Part print with two shaded views. Sizes in mm from the minimum x, y, z corner. A direction names the side the tool comes from. Give positions to 0.01 mm unless a question says otherwise; leave off trailing zeros. Write each loop counter-clockwise with the first axis right and the second up, starting at its lowest first coordinate (ties: lowest second). Pieces come first, ordered by that corner, then holes.
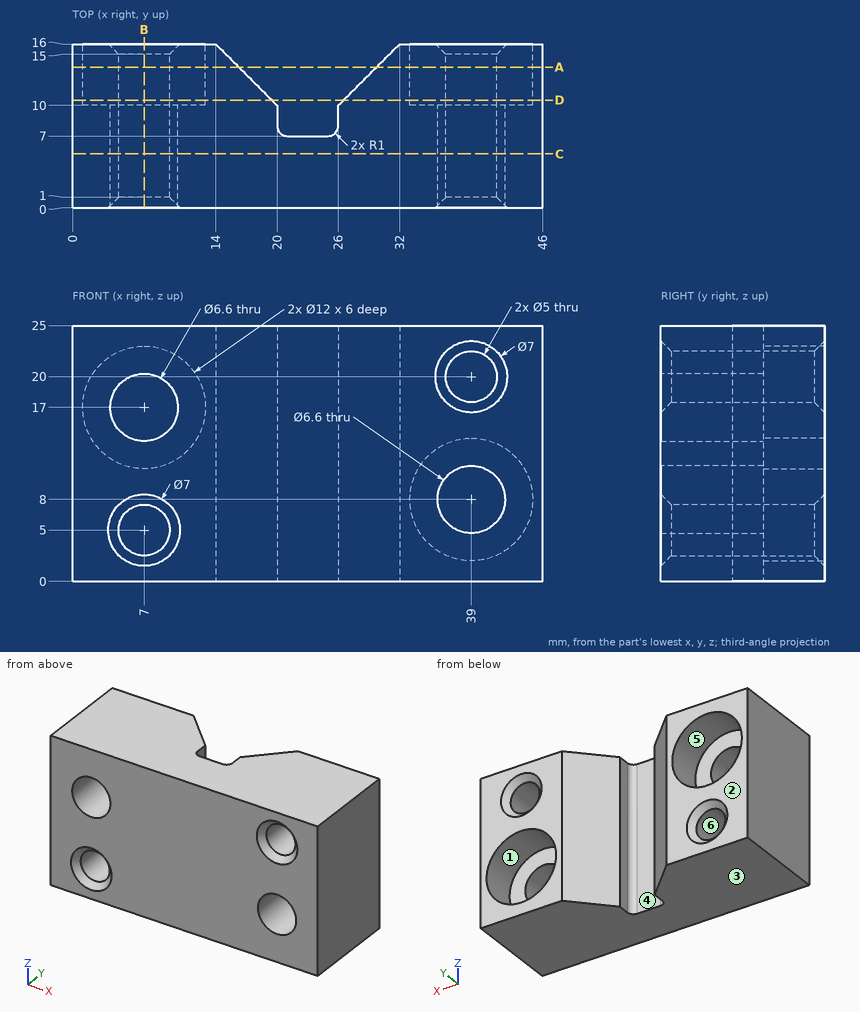
1) Two-plate mould, pull along Z, no slides. Class the marked faces 1, 2 and 3: +Z half, -Z half, draft (parallel to the pull), parting line (faces both ways), or undercut.
Answers follow:
face 1: undercut
face 2: draft
face 3: -Z half
2) Pin check, flat tips, straight feed: pin 1 Ø2 at (x, z) = (23, 14.5) entering from +Y; pin 2 Ø3 at (x, z) = (25.5, 22) entering from +Y; pin 3 Ø6 at (x, z) = (18.5, 4) entering from +Y. Stop position of each tip, or through.
Answers follow:
pin 1: stops at y = 7
pin 2: stops at y = 11
pin 3: stops at y = 14.5
3) Saw through at B-B, the plane x = 7. Write the cut outline in (y, z).
Answers follow:
outline: (0, 0) - (16, 0) - (16, 1.5) - (15, 2.5) - (1, 2.5) - (0, 1.5) - close; (0, 8.5) - (1, 7.5) - (15, 7.5) - (16, 8.5) - (16, 11) - (10, 11) - (10, 13.7) - (0, 13.7) - close; (0, 20.3) - (10, 20.3) - (10, 23) - (16, 23) - (16, 25) - (0, 25) - close
4) Wall check: L1, parallel to X at y = 6.75, z = 20; L2, parallel to X at y = 5, z = 5; L3, parallel to X at y = 8.75, z = 11.5. Give the ranges that are in metal, low to high.
Answers follow:
L1: x = 0 to 5.63, 8.37 to 36.5, 41.5 to 46
L2: x = 0 to 4.5, 9.5 to 37.63, 40.37 to 46
L3: x = 0 to 20, 26 to 46
5) Saw through at C-C, the plane y = 5.25. Write the cut outline in (x, z).
Answers follow:
outline: (0, 0) - (46, 0) - (46, 25) - (0, 25) - close; hole circle Ø6.6 at (7, 17); hole circle Ø5 at (7, 5); hole circle Ø6.6 at (39, 8); hole circle Ø5 at (39, 20)
6) Saw through at D-D, the plane y = 10.5. Write the cut outline in (x, z), then the cut area to 3 significant figures.
Answers follow:
outline: (0, 0) - (19.5, 0) - (19.5, 25) - (0, 25) - close; (26.5, 0) - (46, 0) - (46, 25) - (26.5, 25) - close; hole circle Ø12 at (7, 17); hole circle Ø5 at (7, 5); hole circle Ø12 at (39, 8); hole circle Ø5 at (39, 20)
area: 710 mm2
7) Saw through at A-A, the plane y = 13.75. Write the cut outline in (x, z).
Answers follow:
outline: (0, 0) - (16.25, 0) - (16.25, 25) - (0, 25) - close; (29.75, 0) - (46, 0) - (46, 25) - (29.75, 25) - close; hole circle Ø12 at (7, 17); hole circle Ø5 at (7, 5); hole circle Ø12 at (39, 8); hole circle Ø5 at (39, 20)
8) 3-axis set-ups, long thin cutter, end or side, ignore diameter. For the marked faces 4, 5 and 6: which of +Z, -Z, +X, -X, +Y, -Y reach the whole face in a straight line?
Answers follow:
face 4: +Z, -Z, +Y
face 5: +Y
face 6: +Y, -Y
